from build123d import *

# Parameters (mm, degrees)
SKETCH_1_W                  = 250
SKETCH_1_H                  = 95
EXTRUDE_1_DEPTH             = 10
CUT_EXTRUDE_2_DEPTH         = 135.094183319
PATTERN_LINEAR_1_COUNT      = 2
PATTERN_LINEAR_1_PITCH      = 40
PATTERN_LINEAR_1_COUNT_DIR2 = 2
PATTERN_LINEAR_1_PITCH_DIR2 = 40
PATTERN_LINEAR_2_COUNT      = 2
PATTERN_LINEAR_2_PITCH      = 40
PATTERN_LINEAR_2_COUNT_DIR2 = 2
PATTERN_LINEAR_2_PITCH_DIR2 = 40
CHAMFER_1_SIZE              = 5
HOLE_WIZARD_M10_3_D         = 8.5
HOLE_WIZARD_M10_3_DEPTH     = 24.5
HOLE_WIZARD_M10_3_TIP       = 2.553657631
SKETCH_12_R                 = 13
CUT_EXTRUDE_5_DEPTH         = 135.094183319
HOLE_WIZARD_M4_1_D          = 3.3
HOLE_WIZARD_M4_1_DEPTH      = 10.1
HOLE_WIZARD_M4_1_TIP        = 0.991420021


with BuildPart() as part:
    # 草图1 → 凸台-拉伸1 (new body)
    with BuildSketch(Plane.XY):
        Rectangle(SKETCH_1_W, SKETCH_1_H)
    extrude(amount=EXTRUDE_1_DEPTH)

    # 草图3 → 切除-拉伸2 (cut, through all)
    with BuildSketch(Plane.XY.offset(10)):
        with BuildLine():
            Line((-59.5, -29.5), (-59.5, -25.5))
            ThreePointArc((-59.5, -25.5), (-55, -21), (-50.5, -25.5))
            Line((-50.5, -25.5), (-50.5, -29.5))
            ThreePointArc((-50.5, -29.5), (-55, -34), (-59.5, -29.5))
        make_face()
    cut_extrude_2 = extrude(amount=-CUT_EXTRUDE_2_DEPTH, mode=Mode.SUBTRACT)

    # 阵列(线性)1: Cut-Extrude 2 2 × 2
    with Locations(*[(i * PATTERN_LINEAR_1_PITCH, j * PATTERN_LINEAR_1_PITCH_DIR2, 0) for i in range(PATTERN_LINEAR_1_COUNT) for j in range(PATTERN_LINEAR_1_COUNT_DIR2) if (i, j) != (0, 0)]):
        add(cut_extrude_2, mode=Mode.SUBTRACT)

    # 阵列(线性)2: Cut-Extrude 2 2 × 2
    with Locations(*[(-i * PATTERN_LINEAR_2_PITCH, j * PATTERN_LINEAR_2_PITCH_DIR2, 0) for i in range(PATTERN_LINEAR_2_COUNT) for j in range(PATTERN_LINEAR_2_COUNT_DIR2) if (i, j) != (0, 0)]):
        add(cut_extrude_2, mode=Mode.SUBTRACT)

    # 倒角1
    chamfer_1_edges = [part.edges().sort_by_distance(p)[0] for p in [
        (125, -47.5, 5),
        (-125, -47.5, 5),
        (-125, 47.5, 5),
        (125, 47.5, 5),
    ]]
    chamfer(chamfer_1_edges, length=CHAMFER_1_SIZE)

    # M10 螺纹孔3
    with Locations(Plane(origin=(42.5, 35, 10), x_dir=(1, 0, 0), z_dir=(0, 0, 1))):
        with Locations((0, 0), (70, 0), (70, -70), (0, -70)):
            Hole(HOLE_WIZARD_M10_3_D / 2, depth=HOLE_WIZARD_M10_3_DEPTH)
            with Locations((0, 0, -(HOLE_WIZARD_M10_3_DEPTH + HOLE_WIZARD_M10_3_TIP / 2))):  # 118° drill point
                Cone(0, HOLE_WIZARD_M10_3_D / 2, HOLE_WIZARD_M10_3_TIP, mode=Mode.SUBTRACT)

    # 草图12 → 切除-拉伸5 (cut, through all)
    with BuildSketch(Plane.XY.offset(10)):
        with Locations((77.5, 0)):
            Circle(SKETCH_12_R)
    extrude(amount=-CUT_EXTRUDE_5_DEPTH, mode=Mode.SUBTRACT)

    # M4 螺纹孔1
    with Locations(Plane(origin=(117, -47.5, 5), x_dir=(0, 0, -1), z_dir=(0, -1, 0))):
        with Locations((0, 0), (0, -105), (0, -52.5)):
            Hole(HOLE_WIZARD_M4_1_D / 2, depth=HOLE_WIZARD_M4_1_DEPTH)
            with Locations((0, 0, -(HOLE_WIZARD_M4_1_DEPTH + HOLE_WIZARD_M4_1_TIP / 2))):  # 118° drill point
                Cone(0, HOLE_WIZARD_M4_1_D / 2, HOLE_WIZARD_M4_1_TIP, mode=Mode.SUBTRACT)


solid = part.part
Work out the finished part from the listing and answer in its coordinate system (mm). A direction names the side the tool comes from. Give positions to 0.01 mm unless a question says otherwise; leave off trailing zeros. Write each loop counter-clockwise with the first axis right and the second up, starting at its lowest first coordinate (ties: lowest second). Pieces come first, ordered by that corner, then holes.
Q1. For a pull along Y with two mould halves and no side action, classify faces 1 (the face through (-125, -1, 5)), 2 (the face through (-2, 47.5, 5)), 3 (the face through (-95, 6, 5)), 4 (the face through (64.513, 0.572, 5.07)) as released by +Y, released by -Y, zero draft, split by the parting line, or undercut.
Answer:
face 1: zero draft
face 2: released by +Y
face 3: undercut
face 4: undercut
Q2. The part is cut by section A-A on x = -55. Give the vertices of the cut face in (y, z).
Answer:
outline: (-47.5, 0) - (-34, 0) - (-34, 10) - (-47.5, 10) - close; (-21, 0) - (6, 0) - (6, 10) - (-21, 10) - close; (19, 0) - (47.5, 0) - (47.5, 10) - (19, 10) - close
Q3. The part is cut by section C-C on y = -3. Give the vertices of the cut face in (x, z).
Answer:
outline: (-125, 0) - (64.85, 0) - (64.85, 10) - (-125, 10) - close; (90.15, 0) - (125, 0) - (125, 10) - (90.15, 10) - close
Q4. Straight lines are drawn through the part: L1, parallel to Y at x = -15, z = 1; L2, parallel to Y at x = 112.5, z = 7.25; L3, parallel to X at y = -27.5, z = 6.5. For each, find the intervals that lie inside material, in ascending order.
Answer:
L1: y = -47.5 to -34, -21 to 6, 19 to 47.5
L2: y = -47.5 to -39.25, -30.75 to 30.75, 39.25 to 47.5
L3: x = -125 to -99.5, -90.5 to -59.5, -50.5 to -19.5, -10.5 to 125
Q5. A tool of negligible diameter and unlimited length cuts with its end or side. For faces 5 (the face through (122.5, -45, 4.9)), 6 (the face through (-55, -21, 5)), from which of +Z, -Z, +X, -X, +Y, -Y can it reach the whole face along a straight path? Write none if from no direction.
Answer:
face 5: +Z, -Z, +X, -Y
face 6: +Z, -Z
Q6. The part is cut by section B-B on x = 77.5. Give the vertices of the cut face in (y, z).
Answer:
outline: (-47.5, 0) - (-13, 0) - (-13, 10) - (-47.5, 10) - close; (13, 0) - (47.5, 0) - (47.5, 10) - (13, 10) - close
